```python
from build123d import *

# Parameters (mm, degrees)
SKETCH1_W                   = 80
SKETCH1_H                   = 120
BOSS_EXTRUDE1_DEPTH         = 10
SKETCH2_W                   = 530
SKETCH2_H                   = 110
BOSS_EXTRUDE2_DEPTH         = 12
CHAMFER1_SIZE               = 10
CUT_EXTRUDE1_DEPTH          = 303.553620593
CUT_EXTRUDE1_DEPTH_BACK     = 303.553620593
SKETCH3_R                   = 2.1
M5_TAPPED_HOLE1_D           = 4.2
M5_TAPPED_HOLE1_DEPTH       = 12.4
M5_TAPPED_HOLE1_CSINK_D     = 5.05
M5_TAPPED_HOLE1_CSINK_ANGLE = 90
M5_TAPPED_HOLE1_TIP         = 1.2618073
M8_TAPPED_HOLE1_D           = 6.8
M8_TAPPED_HOLE1_DEPTH       = 22.25
M8_TAPPED_HOLE1_CSINK_D     = 8.05
M8_TAPPED_HOLE1_CSINK_ANGLE = 90
M8_TAPPED_HOLE1_TIP         = 2.042926105


with BuildPart() as part:
    # Sketch1 → Boss-Extrude1 (new body)
    with BuildSketch(Plane(origin=(0, 0, 0), x_dir=(1, 0, 0), z_dir=(0, 1, 0))):
        with Locations((-10, -38.967082208)):
            Rectangle(SKETCH1_W, SKETCH1_H)
    extrude(amount=BOSS_EXTRUDE1_DEPTH)

    # Sketch2 → Boss-Extrude2 (add)
    with BuildSketch(Plane.XY.offset(98.967082208)):
        with Locations((-10, 5)):
            Rectangle(SKETCH2_W, SKETCH2_H)
    extrude(amount=BOSS_EXTRUDE2_DEPTH)

    # Chamfer1
    chamfer1_edges = [part.edges().sort_by_distance(p)[0] for p in [
        (-50, 5, -21.032917792),
        (30, 5, -21.032917792),
    ]]
    chamfer(chamfer1_edges, length=CHAMFER1_SIZE)

    # Sketch3 → Cut-Extrude1 (cut, two sides: drawn at the far end of the back side and taken through both)
    with BuildSketch(Plane(origin=(0, 10, 0), x_dir=(1, 0, 0), z_dir=(0, 1, 0)).offset(-CUT_EXTRUDE1_DEPTH_BACK)):
        with Locations(Location((6.617009358, 0.14992715, 0), (0, 0, 270))):
            Circle(SKETCH3_R)
        with Locations(Location((13.499999853, -16.467082208, 0), (0, 0, 270))):
            Circle(SKETCH3_R)
        with Locations(Location((6.617009358, -33.084091566, 0), (0, 0, 270))):
            Circle(SKETCH3_R)
        with Locations(Location((-26.617009358, -33.084091566, 0), (0, 0, 270))):
            Circle(SKETCH3_R)
        with Locations(Location((-33.499999853, -16.467082208, 0), (0, 0, 270))):
            Circle(SKETCH3_R)
        with Locations(Location((-26.617009358, 0.14992715, 0), (0, 0, 270))):
            Circle(SKETCH3_R)
    extrude(amount=CUT_EXTRUDE1_DEPTH + CUT_EXTRUDE1_DEPTH_BACK, mode=Mode.SUBTRACT)

    # M5 Tapped Hole1
    with Locations(Plane.XY.offset(110.967082208)):
        with Locations((-261.5, 25), (-261.5, -15), (-208.5, 25), (-208.5, -15), (188.5, -15), (188.5, 25), (241.5, -15), (241.5, 25)):
            CounterSinkHole(M5_TAPPED_HOLE1_D / 2, M5_TAPPED_HOLE1_CSINK_D / 2, depth=M5_TAPPED_HOLE1_DEPTH, counter_sink_angle=M5_TAPPED_HOLE1_CSINK_ANGLE)
            with Locations((0, 0, -(M5_TAPPED_HOLE1_DEPTH + M5_TAPPED_HOLE1_TIP / 2))):  # 118° drill point
                Cone(0, M5_TAPPED_HOLE1_D / 2, M5_TAPPED_HOLE1_TIP, mode=Mode.SUBTRACT)

    # M8 Tapped Hole1
    with Locations(Plane.XY.offset(110.967082208)):
        with Locations((-160, 32.5), (-160, -32.5), (140, 32.5), (140, -32.5)):
            CounterSinkHole(M8_TAPPED_HOLE1_D / 2, M8_TAPPED_HOLE1_CSINK_D / 2, depth=M8_TAPPED_HOLE1_DEPTH, counter_sink_angle=M8_TAPPED_HOLE1_CSINK_ANGLE)
            with Locations((0, 0, -(M8_TAPPED_HOLE1_DEPTH + M8_TAPPED_HOLE1_TIP / 2))):  # 118° drill point
                Cone(0, M8_TAPPED_HOLE1_D / 2, M8_TAPPED_HOLE1_TIP, mode=Mode.SUBTRACT)


solid = part.part
```
Input: part model. Units: mm. Frame: model coordinates. A direction names the side the tool comes from. Coordinates: 2 decimals unless noted, no trailing zeros. Loops run counter-clockwise (first coordinate to the right, second up) from the corner with the lowest first, then second, coordinate; pieces in that order, holes last. Notation, with made-up numbers: M 59.25,66 L 83.25,66 A14 cw 83.25,80 Z; hole C -15.75,-26 d7. An arc over 180 degrees is marked long. One line per item, written item: value.
(1) Line query: line 1 along X through (y, z) = (-15, 106); line 2 along Y through (x, z) = (-208.5, 102.25); line 3 along Y through (x, z) = (-160, 106.5). Output: solid intervals per line, ascending. Write a range as from..to.
Filled in:
line 1: -275..-263.6, -259.4..-210.6, -206.4..186.4, 190.6..239.4, 243.6..255
line 2: -50..-17.1, -12.9..22.9, 27.1..60
line 3: -50..-35.9, -29.1..29.1, 35.9..60
(2) Reachability of faces 4 (the flat face through (-11, 0, 38)), 5 (the flat face through (-11, 10, 38)), 6 (the flat face through (-50, 5, 45)) from +Z, -Z, +X, -X, +Y, -Y: full face, straight path, thin tool, end or side. Return the list, or none.
Filled in:
face 4: -Z, +X, -X, -Y
face 5: -Z, +X, -X, +Y
face 6: -Z, -X, +Y, -Y
(3) Pin query (flat end, axial travel): pin 1 (6.5 mm diameter, centred on x = -33.5, z = 16.47, fed in from -Y); pin 2 (5.5 mm diameter, centred on x = 188.5, y = 25, fed in from -Z); pin 3 (6.5 mm diameter, centred on x = -26.62, z = -0.15, fed in from +Y). Return the tip coordinate at first contact, or that it passes through.
Filled in:
pin 1: y = 0
pin 2: z = 98.97
pin 3: y = 10
(4) Section A-A (z = 24.5). Output: boundary loops of the cut face in (x, y).
Filled in:
outline: M -50,0 L 30,0 L 30,10 L -50,10 Z
(5) Section B-B (y = 48.5). Output: boundary loops of the cut face in (x, z), and give its area (3 significant figures).
Filled in:
outline: M -275,98.97 L 255,98.97 L 255,110.97 L -275,110.97 Z
area: 6,360 mm^2
(6) Pull-direction query (Z, two-part tool) for faces 1 (the flat face through (-14, 6, 110.967)), 2 (the flat face through (30, 5, 45)), 3 (the flat face through (-10, 5, -21.033)); classes: +Z half, -Z half, draft (parallel to the pull), parting line (faces both ways), or undercut.
Filled in:
face 1: +Z half
face 2: draft
face 3: -Z half
